Here's the drawing with two shaded views (mm, measured from the low corner). I have some questions. A direction names the side the tool comes from. Round coordinates to 2 decimals unless told otherwise and drop trailing zeros. Order: outer loops, then holes, each group sorted by start corner. A loop starts at its lowest first (then second) coordinate and runs counter-clockwise, first axis right, second up.
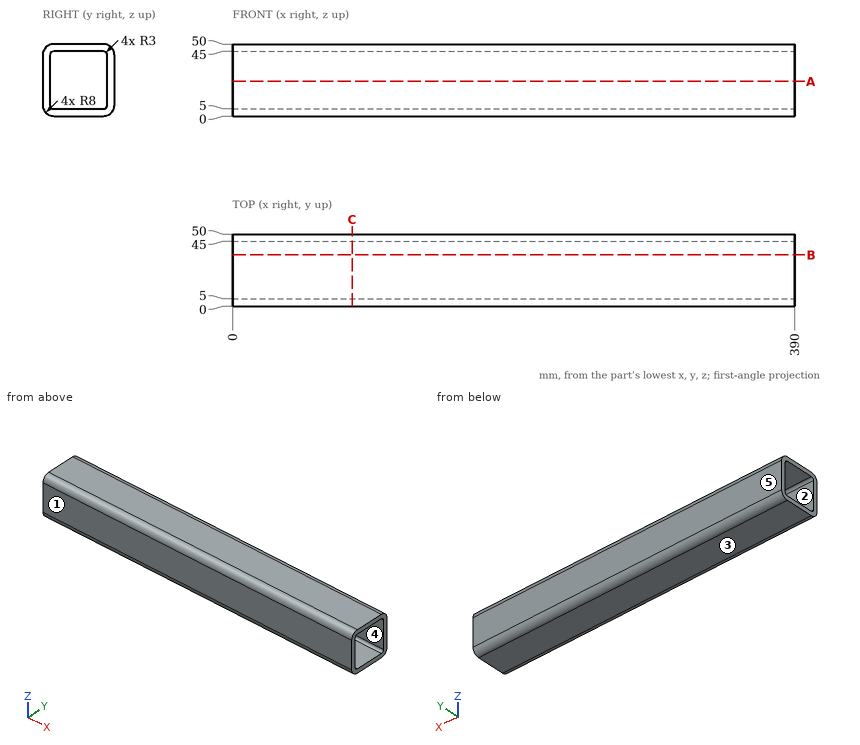
1. If we mould it in two halves opening along Z, with no side actions, what happens to the marked faces 1, 2 and 3? For each: released by +Z, released by -Z, zero draft, split by the parting line, or undercut.
Evaluation:
face 1: zero draft
face 2: undercut
face 3: released by -Z
2. I need wall thicknesses on probe 1 along Z at (x, y) = (235.5, 38.5); probe 2 along Y at (x, z) = (291, 7). Which ranges of each line are inside material? Lowest first, please.
Evaluation:
probe 1: z = 0 to 5, 45 to 50
probe 2: y = 0.06 to 5.17, 44.83 to 49.94
3. If we section it at A-A, the plane z = 24: Write out the boundary of the cut face in (x, y).
Evaluation:
outline: (0, 0) - (390, 0) - (390, 5) - (0, 5) - close; (0, 45) - (390, 45) - (390, 50) - (0, 50) - close
4. On a 3-axis mill with a long thin cutter (end or side, diameter ignored), from which of +Z, -Z, +X, -X, +Y, -Y can I reach the whole of each face in a straight line? I mean the marked faces 4 and 5. Say none if no direction works.
Evaluation:
face 4: +X, -X
face 5: +Z, -Z, +X, -X, +Y
5. If we section it at C-C, the plane x = 83: Write out the boundary of the cut face in (y, z), and give its area (3 significant figures).
Evaluation:
outline: (0, 8) arc R8 ccw to (8, 0) - (42, 0) arc R8 ccw to (50, 8) - (50, 42) arc R8 ccw to (42, 50) - (8, 50) arc R8 ccw to (0, 42) - close; hole (5, 8) arc R3 ccw to (8, 5) - (42, 5) arc R3 ccw to (45, 8) - (45, 42) arc R3 ccw to (42, 45) - (8, 45) arc R3 ccw to (5, 42) - close
area: 853 mm2
6. I'm going to push a flat-ended pin straight in: P1, Ø4, axis at x = 312, z = 19.5, coming from the -Y side. Where does the tip first touch, or does it pass through?
Evaluation:
P1: stops at y = 0
